```python
from build123d import *

# Parameters (mm, degrees)
EXTRUDE_1_DEPTH = 100
FILLET_1_R      = 5


with BuildPart() as part:
    # 草图1 → 凸台-拉伸1 (new body)
    with BuildSketch(Plane(origin=(0, 0, 0), x_dir=(1, 0, 0), z_dir=(0, 1, 0))):
        Polygon((3, 0), (3, 198.267949192), (6.92820323, 200.535898385), (3.92820323, 205.732050808), (-3, 201.732050808), (-3, 0), align=None)
    extrude(amount=EXTRUDE_1_DEPTH)

    # 圆角1
    fillet_1_edges = [part.edges().sort_by_distance(p)[0] for p in [
        (-3, 50, -201.732050808),
    ]]
    fillet(fillet_1_edges, radius=FILLET_1_R)


solid = part.part
```
Source: CAD feature listing. Evaluate the final solid. Frame: model axes, mm. A direction names the side the tool comes from. Round coordinates to 2 decimals unless told otherwise and drop trailing zeros. Loops run counter-clockwise (first coordinate to the right, second up) from the corner with the lowest first, then second, coordinate; pieces in that order, holes last.
(1) Access query for faces 1 (the flat face through (3, 49, -98)), 2 (the flat face through (0, 49, 0)). Directions: +Z, -Z, +X, -X, +Y, -Y. A direction counts if a zero-diameter tool reaches every point of the face in a straight line with its end or side. Return the directions, or none.
From the geometry:
face 1: +Z, +X, +Y, -Y
face 2: +Z, +X, -X, +Y, -Y
(2) Section query B-B (z = -181.5). Output: boundary loops of the cut face in (x, y), and give its area (3 significant figures).
From the geometry:
outline: (-3, 0) - (3, 0) - (3, 100) - (-3, 100) - close
area: 600 mm2
(3) Section query A-A (y = 37). Output: boundary loops of the cut face in (x, z), and give its area (3 significant figures).
From the geometry:
outline: (-3, -198.85) arc R5 ccw to (-0.5, -203.18) - (3.93, -205.73) - (6.93, -200.54) - (3, -198.27) - (3, 0) - (-3, 0) - close
area: 1,240 mm2
(4) Material intervals for probe 1 along X at (y, z) = (33, -99); probe 2 along Z at (x, y) = (-0.5, 93); probe 3 along Z at (x, y) = (-1, 76), sorted ascending.
From the geometry:
probe 1: x = -3 to 3
probe 2: z = -203.18 to 0
probe 3: z = -202.85 to 0
(5) Contact query for flat-ended pins moving along their axis: pin 1 Ø4 at (x, y) = (2.5, 47) entering from -Z; pin 2 Ø3 at (y, z) = (87, -99.5) entering from +X; pin 3 Ø5 at (x, z) = (2.5, -137) entering from -Y; pin 4 Ø3 at (x, y) = (-0.5, 43.5) entering from -Z. Output: stop coordinate, or through.
From the geometry:
pin 1: stops at z = -205.73
pin 2: stops at x = 3
pin 3: stops at y = 0
pin 4: stops at z = -204.04
